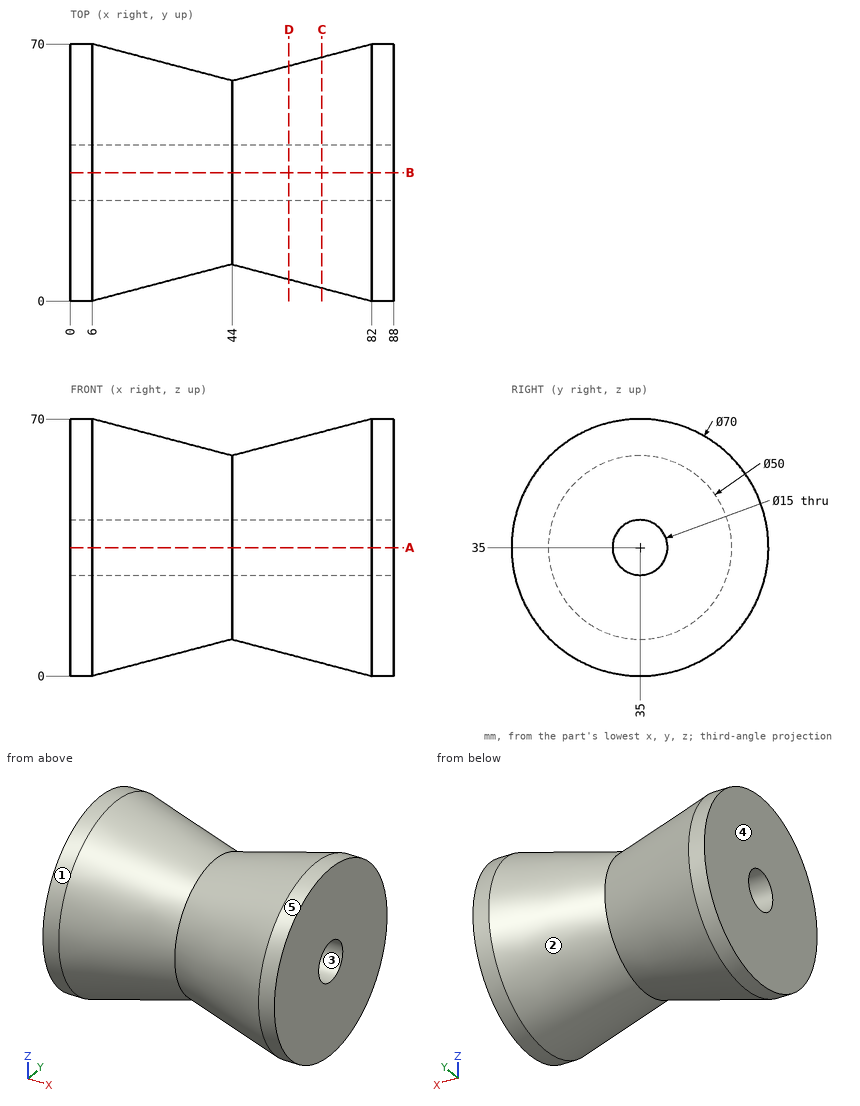
Print and shaded views of the part. All mm, measured from the part's lowest x, y and z. A direction names the side the tool comes from. Coordinates: 2 decimals unless noted, no trailing zeros. Loops run counter-clockwise (first coordinate to the right, second up) from the corner with the lowest first, then second, coordinate; pieces in that order, holes last. Notation, with made-up numbers: (4.5, -2.5) - (45.5, -2.5) arc R18 cw to (45.5, 31.5) - close; hole circle Ø10 at (-22.5, 61). An arc over 180 degrees is marked (long way). Write item = value, one per line. Start each with the question number.
Item 1: Cut at C-C, the plane x = 68.5. Give the cut face in (y, z), and give its area (3 significant figures).
Item 2: Mould opens along Z. For the marked faces 3, 4 and 5 say: released by +Z, released by -Z, zero draft, split by the parting line, or undercut.
Item 3: Cut at D-D, the plane x = 59.5. Give the cut face in (y, z), and give its area (3 significant figures).
Item 4: Flat gauge pins, fed straight in: pin 1 Ø8 at (x, y) = (21, 41) entering from -Z; pin 2 Ø1 at (y, z) = (36.5, 46) entering from -X; pin 3 Ø12 at (x, y) = (36.5, 48) entering from -Z; pin 4 Ø3 at (x, z) = (9, 9.5) entering from -Y. Where does each tip first touch, or does it go through?
Item 5: 3-axis set-ups, long thin cutter, end or side, ignore diameter. For the marked faces 1 and 2: which of +Z, -Z, +X, -X, +Y, -Y reach the whole face in a straight line?
Item 6: Wall check: L1, parallel to Y at x = 66, z = 35; L2, parallel to Z at x = 24, y = 35; L3, parallel to Y at x = 64.5, z = 32. Give the ranges that are in metal, low to high. Write a range as from..to.
Item 7: Cut at A-A, the plane z = 35. Give the cut face in (x, y), and give its area (3 significant figures).
The answers:
q1.outline = circle Ø62.89 at (35, 35); hole circle Ø15 at (35, 35)
q1.area = 2,930 mm2
q2.face_3 = undercut
q2.face_4 = zero draft
q2.face_5 = split by the parting line
q3.outline = circle Ø58.16 at (35, 35); hole circle Ø15 at (35, 35)
q3.area = 2,480 mm2
q4.pin_1 = 3.28
q4.pin_2 = 0
q4.pin_3 = 8.3
q4.pin_4 = 10.52
q5.face_1 = +X, -X
q5.face_2 = none
q6.L1 = 4.21..27.5, 42.5..65.79
q6.L2 = 4.74..27.5, 42.5..65.26
q6.L3 = 4.75..28.13, 41.87..65.25
q7.outline = (0, 0) - (6, 0) - (44, 10) - (82, 0) - (88, 0) - (88, 27.5) - (0, 27.5) - close; (0, 42.5) - (88, 42.5) - (88, 70) - (82, 70) - (44, 60) - (6, 70) - (0, 70) - close
q7.area = 4,080 mm2
